Here's how the part is built. I have some questions about the finished solid (model axes, mm). Face numbers are marked on the shaded views. Give positions to 0.01 mm unless a question says otherwise; leave off trailing zeros. Write each loop counter-clockwise with the first axis right and the second up, starting at its lowest first coordinate (ties: lowest second). Pieces come first, ordered by that corner, then holes. Notation, with made-up numbers: (44, 18) - (56, 18) arc R13 cw to (56, 43) - close; hole circle Ø7 at (74, 54.25). An arc over 180 degrees is marked (long way). Use a Markdown table: item, result.
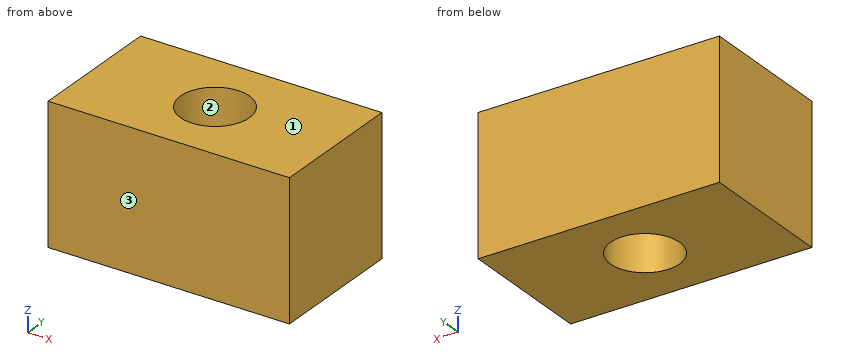
```python
from build123d import *

# Parameters (mm, degrees)
SKETCH1_W           = 35
SKETCH1_H           = 20
SKETCH1_R           = 5
BOSS_EXTRUDE1_DEPTH = 20


with BuildPart() as part:
    # Sketch1 → Boss-Extrude1 (new body)
    with BuildSketch(Plane.XY):
        Rectangle(SKETCH1_W, SKETCH1_H)
        Circle(SKETCH1_R, mode=Mode.SUBTRACT)
    extrude(amount=BOSS_EXTRUDE1_DEPTH)


solid = part.part
```
Item 1: Will this pin go through, and if not, where does the flat tip stop? pin 1 Ø4 at (x, y) = (-12, 2.5) entering from -Z.
Values:
| item | result |
|---|---|
| pin 1 | stops at z = 0 |
Item 2: If we section it at A-A, the plane y = 0: Write out the boundary of the cut face in (x, z), plus the area to 3 significant figures.
Values:
| item | result |
|---|---|
| outline | (-17.5, 0) - (-5, 0) - (-5, 20) - (-17.5, 20) - close; (5, 0) - (17.5, 0) - (17.5, 20) - (5, 20) - close |
| area | 500 mm2 |
Item 3: If we section it at B-B, the plane x = 0: Write out the boundary of the cut face in (y, z).
Values:
| item | result |
|---|---|
| outline | (-10, 0) - (-5, 0) - (-5, 20) - (-10, 20) - close; (5, 0) - (10, 0) - (10, 20) - (5, 20) - close |
Item 4: Thinking about a two-plate mould opening in Y: for the marked faces 1, 2 and 3, which applies, +Y half, -Y half, draft (parallel to the pull), parting line (faces both ways), or undercut?
Values:
| item | result |
|---|---|
| face 1 | draft |
| face 2 | undercut |
| face 3 | -Y half |
Item 5: If we section it at C-C, the plane z = 14.25: Write out the boundary of the cut face in (x, y).
Values:
| item | result |
|---|---|
| outline | (-17.5, -10) - (17.5, -10) - (17.5, 10) - (-17.5, 10) - close; hole circle Ø10 at (0, 0) |
Item 6: I need wall thicknesses on line 1 along X through (y, z) = (0.5, 4); line 2 along Y through (x, z) = (0, 6); line 3 along X through (y, z) = (2, 3.5). Which ranges of each line are inside material? Lowest first, please. Write a range as [from, to].
Values:
| item | result |
|---|---|
| line 1 | x = [-17.5, -4.97], [4.97, 17.5] |
| line 2 | y = [-10, -5], [5, 10] |
| line 3 | x = [-17.5, -4.58], [4.58, 17.5] |
